Read the model definition and answer for the solid it produces. Units are mm, in the model's axes. Face numbers are marked on the shaded views. A direction names the side the tool comes from. Round coordinates to 2 decimals unless told otherwise and drop trailing zeros. Order: outer loops, then holes, each group sorted by start corner. A loop starts at its lowest first (then second) coordinate and runs counter-clockwise, first axis right, second up. Notation, with made-up numbers: M -10,31 L 39,31 A13 ccw 39,40 Z; hole C -31.75,-21.5 d11. An arc over 180 degrees is marked long. Answer as CSV lines item,"result".
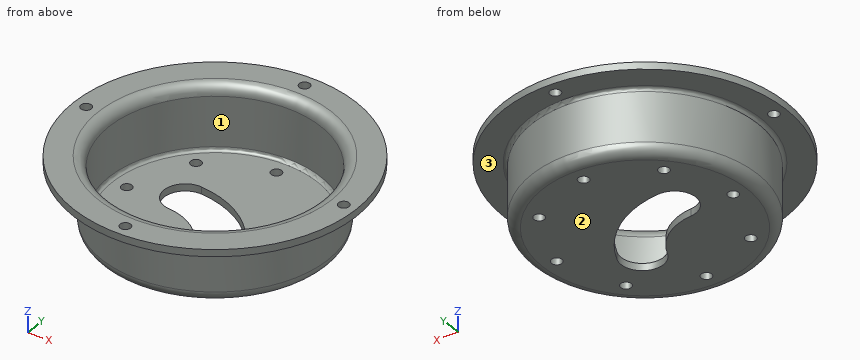
```python
from build123d import *

# Parameters (mm, degrees)
SKETCH1_R           = 160
SKETCH1_R_2         = 7.5
BOSS_EXTRUDE1_DEPTH = 10
SKETCH2_R           = 160
SKETCH2_R_2         = 150
BOSS_EXTRUDE2_DEPTH = 80
SKETCH3_R           = 200
SKETCH3_R_2         = 150
SKETCH3_R_3         = 7.5
BOSS_EXTRUDE3_DEPTH = 10
FILLET1_R           = 5
FILLET2_R           = 15


with BuildPart() as part:
    # Sketch1 → Boss-Extrude1 (new body)
    with BuildSketch(Plane.XY):
        Circle(SKETCH1_R)
        with Locations((0, 125)):
            Circle(SKETCH1_R_2, mode=Mode.SUBTRACT)
        with Locations((88.388347648, 88.388347648)):
            Circle(SKETCH1_R_2, mode=Mode.SUBTRACT)
        with Locations((125, 0)):
            Circle(SKETCH1_R_2, mode=Mode.SUBTRACT)
        with Locations((88.388347648, -88.388347648)):
            Circle(SKETCH1_R_2, mode=Mode.SUBTRACT)
        with Locations((0, -125)):
            Circle(SKETCH1_R_2, mode=Mode.SUBTRACT)
        with Locations((-88.388347648, -88.388347648)):
            Circle(SKETCH1_R_2, mode=Mode.SUBTRACT)
        with Locations((-125, 0)):
            Circle(SKETCH1_R_2, mode=Mode.SUBTRACT)
        with Locations((-88.388347648, 88.388347648)):
            Circle(SKETCH1_R_2, mode=Mode.SUBTRACT)
        with BuildLine():
            ThreePointArc((-53.803098946, 50.037724546), (-86.000050805, 22.408821364), (-58.371147623, -9.788130495))
            ThreePointArc((-58.371147623, -9.788130495), (-17.190203431, -25.016114851), (9.751908775, -59.684317313))
            ThreePointArc((9.751908775, -59.684317313), (48.783936726, -76.312630338), (65.412249751, -37.280602387))
            ThreePointArc((65.412249751, -37.280602387), (18.26355339, 23.388751922), (-53.803098946, 50.037724546))
        make_face(mode=Mode.SUBTRACT)
    extrude(amount=BOSS_EXTRUDE1_DEPTH)

    # Sketch2 → Boss-Extrude2 (add)
    with BuildSketch(Plane.XY.offset(10)):
        Circle(SKETCH2_R)
        Circle(SKETCH2_R_2, mode=Mode.SUBTRACT)
    extrude(amount=BOSS_EXTRUDE2_DEPTH)

    # Sketch3 → Boss-Extrude3 (add)
    with BuildSketch(Plane.XY.offset(90)):
        Circle(SKETCH3_R)
        Circle(SKETCH3_R_2, mode=Mode.SUBTRACT)
        with Locations((0, 182.5)):
            Circle(SKETCH3_R_3, mode=Mode.SUBTRACT)
        with Locations((182.5, 0)):
            Circle(SKETCH3_R_3, mode=Mode.SUBTRACT)
        with Locations((0, -182.5)):
            Circle(SKETCH3_R_3, mode=Mode.SUBTRACT)
        with Locations((-182.5, 0)):
            Circle(SKETCH3_R_3, mode=Mode.SUBTRACT)
    extrude(amount=BOSS_EXTRUDE3_DEPTH)

    # Fillet1
    fillet1_edges = [part.edges().sort_by_distance(p)[0] for p in [
        (-150, 0, 10),
        (-160, 0, 90),
    ]]
    fillet(fillet1_edges, radius=FILLET1_R)

    # Fillet2
    fillet2_edges = [part.edges().sort_by_distance(p)[0] for p in [
        (-160, 0, 0),
        (-150, 0, 100),
    ]]
    fillet(fillet2_edges, radius=FILLET2_R)


solid = part.part
```
Item 1: Flat-ended cylindrical pins translate along their axes: pin 1 (24 mm diameter, centred on x = 88.39, y = 88.39, fed in from +Z); pin 2 (1.5 mm diameter, centred on x = 133, z = 78, fed in from +Y); pin 3 (4 mm diameter, centred on x = -150, z = 29, fed in from -Y). Find the tip coordinate at first contact, or state that the pin passes through.
Ans:
pin 1,"z = 10"
pin 2,"y = 90.06"
pin 3,"y = -60.79"
Item 2: A cutting plane is placed at B-B, the plane z = 30. Determine the outline of the cut face in (x, y).
Ans:
outline,"C 0,0 d320; hole C 0,0 d300"
Item 3: A tool of negligible diameter and unlimited length cuts with its end or side. For the marked faces 1, 2 and 3, from which of +Z, -Z, +X, -X, +Y, -Y can it reach the whole face along a straight path? Write none if from no direction.
Ans:
face 1,"+Z"
face 2,"-Z, +X, -X, +Y, -Y"
face 3,"-Z"
Item 4: Find the intervals of material crossed by probe 1 along X at (y, z) = (-3, 76); probe 2 along Y at (x, z) = (-83, 8.5); probe 3 along Z at (x, y) = (-79, -107), in increasing order. Write a range as [from, to].
Ans:
probe 1,"[-159.97, -149.97], [149.97, 159.97]"
probe 2,"[-135.05, -93.61], [-83.17, 6.87], [33.38, 83.17], [93.61, 135.05]"
probe 3,"[0, 10]"
Item 5: A cutting plane is placed at C-C, the plane y = 0. Give the number of separate pieces and of enclosed holes in the cut face, and give its area (3 significant figures).
Ans:
separate pieces,"6"
enclosed holes,"0"
area,"3,810 mm2"
Item 6: A cutting plane is placed at A-A, the plane x = 182.5. Determine the outline of the cut face in (y, z).
Ans:
outline,"M -81.82,90 L -7.5,90 L -7.5,100 L -81.82,100 Z; M 7.5,90 L 81.82,90 L 81.82,100 L 7.5,100 Z"
